```python
from build123d import *

# Parameters (mm, degrees)
SKETCH2_OUTSIDE_W   = 34.178
SKETCH2_OUTSIDE_H   = 34.178
SKETCH2_OUTSIDE_W_2 = 19.5
SKETCH2_OUTSIDE_H_2 = 19.5
CUT_EXTRUDE1_DEPTH  = 19.733392645
SKETCH3_R           = 1.35
CUT_EXTRUDE2_DEPTH  = 10


with BuildPart() as part:
    # Sketch1 → Revolve1 (revolve)
    with BuildSketch(Plane.XY, mode=Mode.PRIVATE) as revolve1_sk:
        Polygon((5.8, 0), (7.7, 0), (8, 0.3), (8, 4.7), (12.2, 4.7), (12.5, 5), (12.5, 5.9), (12.2, 6.2), (6.8, 6.2), (6.5, 5.9), (6.5, 1.2), (5.8, 1.2), (5.5, 0.9), (5.5, 0.3), align=None)
    revolve(revolve1_sk.sketch.rotate(Axis((0, 0, 0), (0, 1, 0)), 90), axis=Axis((0, 0, 0), (0, 1, 0)))

    # Sketch2 outside → Cut-Extrude1 (cut, through all)
    with BuildSketch(Plane(origin=(0, 6.2, 0), x_dir=(1, 0, 0), z_dir=(0, 1, 0))):
        Rectangle(SKETCH2_OUTSIDE_W, SKETCH2_OUTSIDE_H)
        Rectangle(SKETCH2_OUTSIDE_W_2, SKETCH2_OUTSIDE_H_2, mode=Mode.SUBTRACT)
    extrude(amount=-CUT_EXTRUDE1_DEPTH, mode=Mode.SUBTRACT)

    # Sketch3 → Cut-Extrude2 (cut)
    with BuildSketch(Plane(origin=(0, 6.2, 0), x_dir=(1, 0, 0), z_dir=(0, 1, 0))):
        with Locations(Location((-7.25, 7.25, 0), (0, 0, 270))):
            Circle(SKETCH3_R)
        with Locations(Location((7.25, 7.25, 0), (0, 0, 90))):
            Circle(SKETCH3_R)
        with Locations(Location((7.25, -7.25, 0), (0, 0, 270))):
            Circle(SKETCH3_R)
        with Locations(Location((-7.25, -7.25, 0), (0, 0, 90))):
            Circle(SKETCH3_R)
    extrude(amount=-CUT_EXTRUDE2_DEPTH, mode=Mode.SUBTRACT)


solid = part.part
```
Work out the finished part from the listing and answer in its coordinate system (mm). A direction names the side the tool comes from. Coordinates: 2 decimals unless noted, no trailing zeros. Order: outer loops, then holes, each group sorted by start corner. A loop starts at its lowest first (then second) coordinate and runs counter-clockwise, first axis right, second up. Notation, with made-up numbers: (58, 14.5) - (94, 14.5) arc R28 ccw to (94, 34.5) - close; hole circle Ø7 at (87, 12). An arc over 180 degrees is marked (long way). Answer as a JSON object with one key per item and string values.
1. Consider line 1 (X direction, y = 5.65, z = -7.25); line 2 (X direction, y = 5.5, z = 4); line 3 (X direction, y = 0.75, z = 0). Determine where each line is inside the solid, lowest interval first.
Output values:
{"line 1": "x = -9.75 to -8.6, -5.9 to 5.9, 8.6 to 9.75", "line 2": "x = -9.75 to -5.12, 5.12 to 9.75", "line 3": "x = -8 to -5.5, 5.5 to 8"}
2. The mould has two halves that part along X. Classify faces 4 (the face through (-8.388, 5.46, 6.524)), 5 (the face through (-8.85, 5.46, 8.83)), 6 (the face through (0, 5, 9.75)): +X half, -X half, draft (parallel to the pull), parting line (faces both ways), or undercut.
Output values:
{"face 4": "undercut", "face 5": "-X half", "face 6": "draft"}
3. Find section B-B on x = 0. Determine the outline of the cut face in (y, z).
Output values:
{"outline": "(0, -7.7) - (0.3, -8) - (4.7, -8) - (4.7, -9.75) - (6.2, -9.75) - (6.2, -6.8) - (5.9, -6.5) - (1.2, -6.5) - (1.2, -5.8) - (0.9, -5.5) - (0.3, -5.5) - (0, -5.8) - close; (0, 5.8) - (0.3, 5.5) - (0.9, 5.5) - (1.2, 5.8) - (1.2, 6.5) - (5.9, 6.5) - (6.2, 6.8) - (6.2, 9.75) - (4.7, 9.75) - (4.7, 8) - (0.3, 8) - (0, 7.7) - close"}
4. Each of these flat-tipped pins is pushed along its axis until it touches: P1, Ø2, axis at x = -3.5, y = 1, coming from the +Z side; P2, Ø3, axis at x = 7.25, z = -7.25, coming from the -Y side; P3, Ø10, axis at x = 1, z = 6, coming from the -Y side. Where does it stop, or does it pass through?
Output values:
{"P1": "stops at z = 7.6", "P2": "stops at y = 4.7", "P3": "stops at y = 0"}
5. Find section A-A on y = 5.25. Determine the outline of the cut face in (x, z).
Output values:
{"outline": "(-9.75, -7.82) arc R12.5 ccw to (-7.82, -9.75) - (7.82, -9.75) arc R12.5 ccw to (9.75, -7.82) - (9.75, 7.82) arc R12.5 ccw to (7.82, 9.75) - (-7.82, 9.75) arc R12.5 ccw to (-9.75, 7.82) - close; hole circle Ø2.7 at (-7.25, -7.25); hole circle Ø2.7 at (-7.25, 7.25); hole circle Ø13 at (0, 0); hole circle Ø2.7 at (7.25, -7.25); hole circle Ø2.7 at (7.25, 7.25)"}
6. A tool of negligible diameter and unlimited length cuts with its end or side. For faces 1 (the face through (0, 1.2, 6)), 2 (the face through (8.85, 5.46, -8.83)), 3 (the face through (7.81, 2.53, 1.73)), from which of +Z, -Z, +X, -X, +Y, -Y can it reach the whole face along a straight path? Write none if from no direction.
Output values:
{"face 1": "+Y", "face 2": "-Z, +X, +Y, -Y", "face 3": "-Y"}
